```python
from build123d import *

# Parameters (mm, degrees)
SKETCH_1_R      = 20
SKETCH_1_R_2    = 15.05
EXTRUDE_1_DEPTH = 18.5
CHAMFER_1_SIZE  = 0.5


with BuildPart() as part:
    # 草图1 → 凸台-拉伸1 (new body)
    with BuildSketch(Plane(origin=(0, 0, 0), x_dir=(0, 0, -1), z_dir=(1, 0, 0))):
        Circle(SKETCH_1_R)
        Circle(SKETCH_1_R_2, mode=Mode.SUBTRACT)
    extrude(amount=EXTRUDE_1_DEPTH)

    # 倒角1
    chamfer_1_edges = [part.edges().sort_by_distance(p)[0] for p in [
        (0, 0, 20),
        (18.5, 0, 20),
        (0, 0, 15.05),
        (18.5, 0, 15.05),
    ]]
    chamfer(chamfer_1_edges, length=CHAMFER_1_SIZE)


solid = part.part
```
CAD build for the part. Positions are in the model's coordinates, mm. Round coordinates to 2 decimals unless told otherwise and drop trailing zeros. Order: outer loops, then holes, each group sorted by start corner. A loop starts at its lowest first (then second) coordinate and runs counter-clockwise, first axis right, second up.
Item 1: Pin check, flat tips, straight feed: pin 1 (10 mm diameter, centred on x = 8, y = -11, fed in from -Z); pin 2 (10 mm diameter, centred on x = 13.5, z = 10.5, fed in from -Y); pin 3 (4 mm diameter, centred on x = 8, y = 16, fed in from +Z). Stop position of each tip, or through.
Item 2: Saw through at A-A on y = 0. Write the cut outline in (x, z), then the cut area to 3 significant figures.
Item 3: Mould opens along Z. For faces 1 (the face through (9.128, -19.524, 4.336)), 2 (the face through (9.128, -14.692, 3.263)), 3 (the face through (0, -9, 13)) say: pulls with the +Z half, pulls with the -Z half, needs draft (parallel to the pull), parting line crosses it, or undercut.
Item 4: Probe line 1 along Y through (x, z) = (6.25, 0); line 2 along Z through (x, y) = (17.75, -13); line 3 along Y through (x, z) = (16, -8.5). List the from-to ranges inside material, lowest first.
Item 5: Saw through at C-C on x = 15.5. Write the cut outline in (y, z).
Reported:
1. pin 1: stops at z = -19.08
1. pin 2: stops at y = -19.23
1. pin 3: stops at z = 14.28
2. outline: (0, -19.5) - (0.5, -20) - (18, -20) - (18.5, -19.5) - (18.5, -15.55) - (18, -15.05) - (0.5, -15.05) - (0, -15.55) - close; (0, 15.55) - (0.5, 15.05) - (18, 15.05) - (18.5, 15.55) - (18.5, 19.5) - (18, 20) - (0.5, 20) - (0, 19.5) - close
2. area: 182 mm2
3. face 1: parting line crosses it
3. face 2: undercut
3. face 3: needs draft
4. line 1: y = -20 to -15.05, 15.05 to 20
4. line 2: z = -15.2 to -7.58, 7.58 to 15.2
4. line 3: y = -18.1 to -12.42, 12.42 to 18.1
5. outline: circle Ø40 at (0, 0); hole circle Ø30.1 at (0, 0)
